```python
from build123d import *

# Parameters (mm, degrees)
CUT_EXTRUDE1_DEPTH = 3


with BuildPart() as part:
    # Logo3_bib1 → Revolve1 (revolve)
    with BuildSketch(Plane(origin=(0, 0, 0), x_dir=(-1, 0, 0), z_dir=(0, -1, 0))):
        with BuildLine():
            Line((0, -25), (0, 8))
            Line((0, 8), (6, 8))
            ThreePointArc((6, 8), (6.353553391, 7.853553391), (6.5, 7.5))
            Line((6.5, 7.5), (6.5, 0))
            Line((6.5, 0), (4, 0))
            Line((4, 0), (4, -0.01))
            Line((4, -0.01), (3.488425636, -0.01))
            ThreePointArc((3.488425636, -0.01), (3.468729481, -0.026527036), (3.481585234, -0.048793852))
            Line((3.481585234, -0.048793852), (4, -0.237481396))
            Line((4, -0.237481396), (4, -24.375))
            Line((4, -24.375), (3.375, -25))
            Line((3.375, -25), (0, -25))
        make_face()
    revolve(axis=Axis((0, 0, -10.585154653), (0, 0, 1)))

    # Logo3_bib2 → Cut-Extrude1 (cut)
    with BuildSketch(Plane(origin=(0, 0, -8), x_dir=(1, 0, 0), z_dir=(0, 0, -1))):
        Polygon((3.464101615, 0), (1.732050808, 3), (-1.732050808, 3), (-3.464101615, 0), (-1.732050808, -3), (1.732050808, -3), align=None)
    extrude(amount=-CUT_EXTRUDE1_DEPTH, mode=Mode.SUBTRACT)


solid = part.part
```
Read the model definition and answer for the solid it produces. Units are mm, in the model's axes. A direction names the side the tool comes from. Give positions to 0.01 mm unless a question says otherwise; leave off trailing zeros. Loops run counter-clockwise (first coordinate to the right, second up) from the corner with the lowest first, then second, coordinate; pieces in that order, holes last.
Item 1: Find the intervals of material crossed by line 1 along Z through (x, y) = (-3.75, -4.5); line 2 along Z through (x, y) = (1.5, 1); line 3 along X through (y, z) = (0.75, 10.5), in increasing order.
Item 2: The part is cut by section B-B (z = 1). Write down the section's boundary in (x, y), and give its area (3 significant figures).
Item 3: Each of these flat-tipped pins is pushed along its axis until it touches: pin 1 Ø3 at (y, z) = (-4.5, 3) entering from +X; pin 2 Ø2 at (x, y) = (-5, -5) entering from -Z; pin 3 Ø1.5 at (x, y) = (-4.5, 3.5) entering from +Z. Where does it stop, or does it pass through?
Item 4: For faces 1 (the flat face through (3, 3, -8)), 2 (the cylindrical face through (0.867, 3.905, 12.475)), 3 (the flat face through (2.6, -1.5, -6.5)), determine the directions among +Z, -Z, +X, -X, +Y, -Y from which every point of the face is accessible in a straight line to the end or side of a thin tool.
Item 5: The part is cut by section A-A (x = 0). Write down the section's boundary in (y, z) (3 decimals), and give its area (3 significant figures).
Taken from the geometry:
1. line 1: z = -8 to 0
1. line 2: z = -5 to 25
1. line 3: x = -3.93 to 3.93
2. outline: circle Ø8 at (0, 0)
2. area: 50.3 mm2
3. pin 1: stops at x = 2.65
3. pin 2: stops at z = -7.99
3. pin 3: stops at z = 0
4. face 1: -Z, +X, -X, +Y, -Y
4. face 2: +Z
4. face 3: -Z
5. outline: (-6.5, -7.5) arc R0.5 ccw to (-6, -8) - (-3, -8) - (-3, -5) - (3, -5) - (3, -8) - (6, -8) arc R0.5 ccw to (6.5, -7.5) - (6.5, 0) - (4, 0) - (4, 0.01) - (3.488, 0.01) arc R0.02 cw to (3.482, 0.049) - (4, 0.237) - (4, 24.375) - (3.375, 25) - (-3.375, 25) - (-4, 24.375) - (-4, 0.237) - (-3.482, 0.049) arc R0.02 cw to (-3.488, 0.01) - (-4, 0.01) - (-4, 0) - (-6.5, 0) - close
5. area: 285 mm2
